CAD build for the part. Positions are in the model's coordinates, mm. Face numbers are marked on the shaded views. A direction names the side the tool comes from. Give positions to 0.01 mm unless a question says otherwise; leave off trailing zeros. Write each loop counter-clockwise with the first axis right and the second up, starting at its lowest first coordinate (ties: lowest second). Pieces come first, ordered by that corner, then holes. Notation, with made-up numbers: (5, 3.25) - (36, 3.25) arc R6 ccw to (36, 7.25) - close; hole circle Ø5 at (-29.5, 48.25). An arc over 180 degrees is marked (long way). Answer as a JSON object with one key per item and string values.
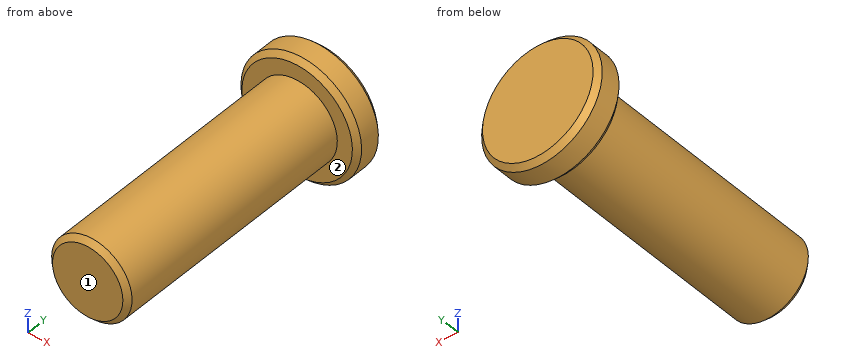
from build123d import *

# Parameters (mm, degrees)
SKETCH2_R           = 4
BOSS_EXTRUDE1_DEPTH = 25
SKETCH3_R           = 6
BOSS_EXTRUDE2_DEPTH = 3
CHAMFER1_SIZE       = 0.5


with BuildPart() as part:
    # Sketch2 → Boss-Extrude1 (new body)
    with BuildSketch(Plane(origin=(0, 0, 0), x_dir=(1, 0, 0), z_dir=(0, 1, 0))):
        with Locations(Location((0, 0, 0), (0, 0, 270))):
            Circle(SKETCH2_R)
    extrude(amount=BOSS_EXTRUDE1_DEPTH)

    # Sketch3 → Boss-Extrude2 (add)
    with BuildSketch(Plane(origin=(0, 25, 0), x_dir=(1, 0, 0), z_dir=(0, 1, 0))):
        with Locations(Location((0, 0, 0), (0, 0, 270))):
            Circle(SKETCH3_R)
    extrude(amount=BOSS_EXTRUDE2_DEPTH)

    # Chamfer1
    chamfer1_edges = [part.edges().sort_by_distance(p)[0] for p in [
        (0, 0, -4),
        (0, 25, -6),
        (0, 28, -6),
    ]]
    chamfer(chamfer1_edges, length=CHAMFER1_SIZE)


solid = part.part
(1) Saw through at C-C, the plane y = 15.75. Give the cut face in (x, z), and give its area (3 significant figures).
Answer key:
{"outline": "circle Ø8 at (0, 0)", "area": "50.3 mm²"}
(2) Probe L1, parallel to Y at x = 2.75, z = 4; L2, parallel to Z at x = 1.25, y = 23. List the from-to ranges inside material, lowest first. Write a range as [from, to].
Answer key:
{"L1": "y = [25, 28]", "L2": "z = [-3.8, 3.8]"}
(3) Saw through at A-A, the plane z = 0. Give the cut face in (x, y).
Answer key:
{"outline": "(-6, 25.5) - (-5.5, 25) - (-4, 25) - (-4, 0.5) - (-3.5, 0) - (3.5, 0) - (4, 0.5) - (4, 25) - (5.5, 25) - (6, 25.5) - (6, 27.5) - (5.5, 28) - (-5.5, 28) - (-6, 27.5) - close"}
(4) 3-axis set-ups, long thin cutter, end or side, ignore diameter. For the marked faces 1 and 2: which of +Z, -Z, +X, -X, +Y, -Y reach the whole face in a straight line?
Answer key:
{"face 1": "+Z, -Z, +X, -X, -Y", "face 2": "-Y"}
(5) Saw through at B-B, the plane x = 0. Give the cut face in (y, z).
Answer key:
{"outline": "(0, -3.5) - (0.5, -4) - (25, -4) - (25, -5.5) - (25.5, -6) - (27.5, -6) - (28, -5.5) - (28, 5.5) - (27.5, 6) - (25.5, 6) - (25, 5.5) - (25, 4) - (0.5, 4) - (0, 3.5) - close"}
(6) Flat gauge pins, fed straight in: P1, Ø2, axis at x = -4, z = -4.5, coming from the -Y side; P2, Ø5, axis at y = 23.5, z = 4.5, coming from the +X side; P3, Ø6, axis at x = -3, y = 11.5, coming from the +Z side. Where does each tip first touch, or does it go through?
Answer key:
{"P1": "stops at y = 25", "P2": "stops at x = 5.2", "P3": "stops at z = 4"}
